```python
from build123d import *

# Parameters (mm, degrees)
SKETCH1_W                                          = 40
SKETCH1_H                                          = 25
BOSS_EXTRUDE1_DEPTH                                = 10
SKETCH2_W                                          = 40
SKETCH2_H                                          = 20
CUT_EXTRUDE1_DEPTH                                 = 2
M5_TAPPED_HOLE1_D                                  = 4.2
HOLE_SIZE_BASED_ON_SOCKET_HEAD_CAP_SCR_D           = 3.4
HOLE_SIZE_BASED_ON_SOCKET_HEAD_CAP_SCR_CBORE_D     = 6
HOLE_SIZE_BASED_ON_SOCKET_HEAD_CAP_SCR_CBORE_DEPTH = 3.4
CHAMFER1_SIZE                                      = 3
CHAMFER2_SIZE                                      = 0.5


with BuildPart() as part:
    # Sketch1 → Boss-Extrude1 (new body)
    with BuildSketch(Plane.XY):
        Rectangle(SKETCH1_W, SKETCH1_H)
    extrude(amount=BOSS_EXTRUDE1_DEPTH)

    # Sketch2 → Cut-Extrude1 (cut)
    with BuildSketch(Plane.XY.offset(10)):
        Rectangle(SKETCH2_W, SKETCH2_H)
    extrude(amount=-CUT_EXTRUDE1_DEPTH, mode=Mode.SUBTRACT)

    # M5 Tapped Hole1 (through all)
    with Locations(Plane.XY.offset(8)):
        with Locations((-15, 0)):
            Hole(M5_TAPPED_HOLE1_D / 2)

    # Hole Size (Based On) Socket Head Cap Screw Type1 (through all)
    with Locations(Plane(origin=(0, 0, 0), x_dir=(-1, 0, 0), z_dir=(0, 0, -1))):
        with Locations((-10, 7.5), (-10, -7.5), (0, 7.5), (0, -7.5)):
            CounterBoreHole(HOLE_SIZE_BASED_ON_SOCKET_HEAD_CAP_SCR_D / 2, HOLE_SIZE_BASED_ON_SOCKET_HEAD_CAP_SCR_CBORE_D / 2, HOLE_SIZE_BASED_ON_SOCKET_HEAD_CAP_SCR_CBORE_DEPTH)

    # Chamfer1
    chamfer1_edges = [part.edges().sort_by_distance(p)[0] for p in [
        (20, -12.5, 5),
        (20, 12.5, 5),
        (-20, -12.5, 5),
        (-20, 12.5, 5),
    ]]
    chamfer(chamfer1_edges, length=CHAMFER1_SIZE)

    # Chamfer2
    chamfer2_edges = [part.edges().sort_by_distance(p)[0] for p in [
        (20, 0, 0),
        (0, -12.5, 0),
        (-20, 0, 0),
        (0, 12.5, 0),
        (0, -12.5, 10),
        (0, 12.5, 10),
    ]]
    chamfer(chamfer2_edges, length=CHAMFER2_SIZE)


solid = part.part
```
Source: CAD feature listing. Evaluate the final solid. Frame: model axes, mm. A direction names the side the tool comes from. Round coordinates to 2 decimals unless told otherwise and drop trailing zeros. Loops run counter-clockwise (first coordinate to the right, second up) from the corner with the lowest first, then second, coordinate; pieces in that order, holes last.
1. Section query A-A on y = 0. Output: boundary loops of the cut face in (x, z), and give its area (3 significant figures).
2. Contact query for flat-ended pins moving along their axis: pin 1 (7 mm diameter, centred on x = 0, y = 7.5, fed in from +Z); pin 2 (3 mm diameter, centred on x = 9.5, y = -7, fed in from -Z); pin 3 (3 mm diameter, centred on x = 10, y = 7.5, fed in from +Z). Output: stop coordinate, or through.
3. Section query D-D on z = 5.5. Output: boundary loops of the cut face in (x, y).
4. Section query C-C on y = -7.5. Output: boundary loops of the cut face in (x, z).
5. Access query for faces 1 (the flat face through (0, -10, 9)), 2 (the cylindrical face through (9.63, -9.16, 5.73)), 3 (the cylindrical face through (12.21, -5.47, 1.68)). Directions: +Z, -Z, +X, -X, +Y, -Y. A direction counts if a zero-diameter tool reaches every point of the face in a straight line with its end or side. Return the directions, or none.
6. Ray query, L1, parallel to Y at x = 0, z = 2.75; L2, parallel to Y at x = 10, z = 4.95; L3, parallel to Y at x = -15, z = 5. Return the intervals inside material, ascending.
7. Section query B-B on x = 10. Output: boundary loops of the cut face in (y, z), and give its area (3 significant figures).
8. Mould query, pull axis X, two halves, no side actions, for faces 4 (the flat face through (0, 0, 8)), 5 (the cylindrical face through (-12.9, 0.09, 3.94)), 6 (the flat face through (-20, 0, 4)). Classes: released by +X, released by -X, zero draft, split by the parting line, or undercut.
Answers below:
1. outline: (-20, 0.5) - (-19.5, 0) - (-17.1, 0) - (-17.1, 8) - (-20, 8) - close; (-12.9, 0) - (19.5, 0) - (20, 0.5) - (20, 8) - (-12.9, 8) - close
1. area: 286 mm2
2. pin 1: stops at z = 10
2. pin 2: stops at z = 3.4
2. pin 3: passes through
3. outline: (-20, -9.5) - (-17, -12.5) - (17, -12.5) - (20, -9.5) - (20, 9.5) - (17, 12.5) - (-17, 12.5) - (-20, 9.5) - close; hole circle Ø4.2 at (-15, 0); hole circle Ø3.4 at (0, -7.5); hole circle Ø3.4 at (0, 7.5); hole circle Ø3.4 at (10, -7.5); hole circle Ø3.4 at (10, 7.5)
4. outline: (-20, 0.5) - (-19.5, 0) - (-3, 0) - (-3, 3.4) - (-1.7, 3.4) - (-1.7, 8) - (-20, 8) - close; (1.7, 3.4) - (3, 3.4) - (3, 0) - (7, 0) - (7, 3.4) - (8.3, 3.4) - (8.3, 8) - (1.7, 8) - close; (11.7, 3.4) - (13, 3.4) - (13, 0) - (19.5, 0) - (20, 0.5) - (20, 8) - (11.7, 8) - close
5. face 1: +Z, +X, -X
5. face 2: +Z, -Z
5. face 3: -Z
6. L1: y = -12.5 to -10.5, -4.5 to 4.5, 10.5 to 12.5
6. L2: y = -12.5 to -9.2, -5.8 to 5.8, 9.2 to 12.5
6. L3: y = -12.5 to -2.1, 2.1 to 12.5
7. outline: (-12.5, 0.5) - (-12, 0) - (-10.5, 0) - (-10.5, 3.4) - (-9.2, 3.4) - (-9.2, 8) - (-10, 8) - (-10, 10) - (-12, 10) - (-12.5, 9.5) - close; (-5.8, 3.4) - (-4.5, 3.4) - (-4.5, 0) - (4.5, 0) - (4.5, 3.4) - (5.8, 3.4) - (5.8, 8) - (-5.8, 8) - close; (9.2, 3.4) - (10.5, 3.4) - (10.5, 0) - (12, 0) - (12.5, 0.5) - (12.5, 9.5) - (12, 10) - (10, 10) - (10, 8) - (9.2, 8) - close
7. area: 137 mm2
8. face 4: zero draft
8. face 5: undercut
8. face 6: released by -X
